For this review, take the finished solid that the model builds, in its own axes (mm). A direction names the side the tool comes from. Coordinates: 2 decimals unless noted, no trailing zeros. Order: outer loops, then holes, each group sorted by start corner. A loop starts at its lowest first (then second) coordinate and runs counter-clockwise, first axis right, second up. Notation, with made-up numbers: (4, 55.25) -> (17, 55.25) arc R26 cw to (17, 78.25) -> close; hole circle Ø7 at (88.5, -35). An arc over 180 degrees is marked (long way). Answer as a JSON object with one key per item and string values. Group by question number.
1) For pin 1 (1.5 mm diameter, centred on x = 3, y = -2.5, fed in from +Z); pin 2 (0.6 mm diameter, centred on y = -3, z = 2.5, fed in from -X); pin 3 (0.8 mm diameter, centred on x = 5, z = 0.5, fed in from +Y); pin 4 (2 mm diameter, centred on x = 8.5, y = -4, fed in from -Z), all flat-tipped, find the tip position at first contact; note any pin that passes through.
2) Draft analysis for pull direction Y (two halves, no side actions). For faces 1 (the flat face through (5, -4, 3)), 2 (the cylindrical face through (9.49, -4.76, 1.97)), 3 (the flat face through (8, -8, 2)), 4 (the flat face through (8, 0, 2)), state which applies: +Y half, -Y half, draft (parallel to the pull), parting line (faces both ways), or undercut.
3) Wall thickness on L1, parallel to Y at x = 8.5, z = 1.05; L2, parallel to Z at x = 3.25, y = -1.5; L3, parallel to X at y = -1.25, z = 0.8: over which ranges is each line inside the solid? List them lowest first.
4) Add section D-D, the plane y = -3. Write out the cut boundary in (x, z).
5) Add section A-A, the plane y = -4. Write out the cut boundary in (x, z), then the cut area to 3 significant figures.
6) Add section C-C, the plane z = 3.3. Write out the cut boundary in (x, y), then the cut area to 3 significant figures.
7) Add section B-B, the plane x = 8.5. Write out the cut boundary in (y, z).
8) Machinability: for faces 5 (the flat face through (3, -4, 2)), 6 (the flat face through (7, -4, 4)), 7 (the flat face through (4, -3, 1)), which of the approach directions +Z, -Z, +X, -X, +Y, -Y give a long, thin tool a straight path to every point of the face, cutting with its end or side? Answer none if there is none.
from build123d import *

# Parameters (mm, degrees)
SKETCH1_W             = 12
SKETCH1_H             = 8
BOSS_EXTRUDE1_DEPTH   = 2
SKETCH2_W             = 7
SKETCH2_H             = 8
BOSS_EXTRUDE2_DEPTH   = 2
SKETCH3_R             = 1.25
CUT_EXTRUDE1_DEPTH    = 10
CUT_EXTRUDE2_DEPTH    = 1
SKETCH5_W             = 2
SKETCH5_H             = 8
CUT_EXTRUDE3_DEPTH    = 7
MOVE_FACE1_BY         = 0.5
M3_TAPPED_HOLE4_D     = 2.5
M3_TAPPED_HOLE4_DEPTH = 7.5
M3_TAPPED_HOLE4_TIP   = 0.751075774


with BuildPart() as part:
    # Sketch1 → Boss-Extrude1 (new body)
    with BuildSketch(Plane.XY):
        with Locations((6, -4)):
            Rectangle(SKETCH1_W, SKETCH1_H)
    extrude(amount=BOSS_EXTRUDE1_DEPTH)

    # Sketch2 → Boss-Extrude2 (add)
    with BuildSketch(Plane.XY.offset(2)):
        with Locations((8.5, -4)):
            Rectangle(SKETCH2_W, SKETCH2_H)
    extrude(amount=BOSS_EXTRUDE2_DEPTH)

    # Sketch3 → Cut-Extrude1 (cut)
    with BuildSketch(Plane.XY.offset(4)):
        with Locations((8.5, -4)):
            Circle(SKETCH3_R)
    extrude(amount=-CUT_EXTRUDE1_DEPTH, mode=Mode.SUBTRACT)

    # Sketch4 → Cut-Extrude2 (cut)
    with BuildSketch(Plane(origin=(0, 0, 0), x_dir=(-1, 0, 0), z_dir=(0, 0, -1))):
        Polygon((0, -4), (0, 1.17366925), (-6, 1.17366925), (-6, -4), (-6, -6.5), (0, -6.5), align=None)
    extrude(amount=-CUT_EXTRUDE2_DEPTH, mode=Mode.SUBTRACT)

    # Sketch5 → Cut-Extrude3 (cut)
    with BuildSketch(Plane(origin=(0, 0, 0), x_dir=(-1, 0, 0), z_dir=(0, 0, -1))):
        with Locations((-1, -4)):
            Rectangle(SKETCH5_W, SKETCH5_H)
    extrude(amount=-CUT_EXTRUDE3_DEPTH, mode=Mode.SUBTRACT)

    # Move Face1: a curved face moved outward by 0.5
    add(Solid.thicken(part.faces().sort_by_distance((7.25, -4, 2))[0], MOVE_FACE1_BY))

    # M3 Tapped Hole4
    with Locations(Plane.XY.offset(4)):
        with Locations((8.5, -4)):
            Hole(M3_TAPPED_HOLE4_D / 2, depth=M3_TAPPED_HOLE4_DEPTH)
            with Locations((0, 0, -(M3_TAPPED_HOLE4_DEPTH + M3_TAPPED_HOLE4_TIP / 2))):  # 118° drill point
                Cone(0, M3_TAPPED_HOLE4_D / 2, M3_TAPPED_HOLE4_TIP, mode=Mode.SUBTRACT)


solid = part.part
Output values:
{
 "1": {"pin 1": "stops at z = 2", "pin 2": "stops at x = 5", "pin 3": "stops at y = -6.5", "pin 4": "passes through"},
 "2": {"face 1": "draft", "face 2": "undercut", "face 3": "-Y half", "face 4": "+Y half"},
 "3": {"L1": "y = -8 to -5.25, -2.75 to 0", "L2": "z = 1 to 2", "L3": "x = 6 to 12"},
 "4": {"outline": "(2, 1) -> (6, 1) -> (6, 0) -> (7.75, 0) -> (7.75, 4) -> (5, 4) -> (5, 2) -> (2, 2) -> close; (9.25, 0) -> (12, 0) -> (12, 4) -> (9.25, 4) -> close"},
 "5": {"outline": "(2, 1) -> (6, 1) -> (6, 0) -> (7.25, 0) -> (7.25, 4) -> (5, 4) -> (5, 2) -> (2, 2) -> close; (9.75, 0) -> (12, 0) -> (12, 4) -> (9.75, 4) -> close", "area": "20.0 mm²"},
 "6": {"outline": "(5, -8) -> (12, -8) -> (12, 0) -> (5, 0) -> close; hole circle Ø2.5 at (8.5, -4)", "area": "51.1 mm²"},
 "7": {"outline": "(-8, 0) -> (-5.25, 0) -> (-5.25, 4) -> (-8, 4) -> close; (-2.75, 0) -> (0, 0) -> (0, 4) -> (-2.75, 4) -> close"},
 "8": {"face 5": "+Z, -X, +Y, -Y", "face 6": "+Z, +X, -X, +Y, -Y", "face 7": "-Z, -X, +Y"}
}
